Check sheet for the modelled part. Datum: model origin and axes. Units: mm. A direction names the side the tool comes from. Give positions to 0.01 mm unless a question says otherwise; leave off trailing zeros. Write each loop counter-clockwise with the first axis right and the second up, starting at its lowest first coordinate (ties: lowest second). Pieces come first, ordered by that corner, then holes. Notation, with made-up numbers: M 15.5,40 L 71.5,40 A32 cw 71.5,79 Z; hole C 19,48 d9. An arc over 180 degrees is marked long. Write item = value, one per line. Start each with the question number.
1) Sectioned sample at B-B, the plane y = 0. Record the cut outline in (x, z).
2) Scan lines: L1, parallel to Y at x = 0, z = 4.75; L2, parallel to Y at x = -4, z = -32; L3, parallel to Z at x = -3, y = -11.5. Record each from-to range of solid material in increasing order.
3) Gauge pin test, flat ends, axial feed: pin 1 (4 mm diameter, centred on y = -20, z = 0.5, fed in from -X); pin 2 (1.5 mm diameter, centred on y = -0.5, z = 4, fed in from -X); pin 3 (7.5 mm diameter, centred on x = -6, y = -20, fed in from +Z); pin 4 (10 mm diameter, centred on y = -34, z = -3, fed in from +X). Record the tip position at first contact, or that the pin passes through.
4) Set-up check for faces 1 (the face through (0.387, 12.494, 0.14)), 2 (the face through (-0.96, -56.07, 33.86)), 3 (the face through (0, -51, -30)), 4 (the face through (0, -15, 10)), 5 (the face through (10, -41, 1)): record each of +Z, -Z, +X, -X, +Y, -Y from which the full face is reachable in a straight line by a thin tool's end or side.
5) Draft check along Y on faces 6 (the face through (-7.493, 0.33, -0.14)), 7 (the face through (-10, -41, 1)), 8 (the face through (0, -51, 31)). Enter one of: pulls with the +Y half, pulls with the -Y half, needs draft (parallel to the pull), parting line crosses it, or undercut.
6) Sectioned sample at D-D, the plane z = 29.5. Record the cut outline in (x, y).
7) Sectioned sample at C-C, the plane z = 7. Record the cut outline in (x, y), then the cut area to 3 significant figures.
8) Sectioned sample at A-A, the plane x = 0. Record the cut outline in (y, z), then the cut area to 3 significant figures.
from build123d import *

# Parameters (mm, degrees)
SKETCH_1_R           = 12.5
SKETCH_1_R_2         = 7.5
EXTRUDE_1_DEPTH      = 10
EXTRUDE_3_DEPTH      = 10
EXTRUDE_4_REACH      = 66.833
EXTRUDE_4_END_RADIUS = 12.5
SKETCH_6_W           = 20
SKETCH_6_H           = 20
HOLE_WIZARD_M6_1_D   = 5


with BuildPart() as part:
    # Sketch 1 → Extrude 1 (new, symmetric)
    with BuildSketch(Plane.XY):
        Circle(SKETCH_1_R)
        Circle(SKETCH_1_R_2, mode=Mode.SUBTRACT)
    extrude(amount=EXTRUDE_1_DEPTH, both=True)



with BuildPart() as body_2:
    # Sketch 5 → Extrude 3 (new, symmetric)
    with BuildSketch(Plane(origin=(0, 0, 0), x_dir=(0, 0, -1), z_dir=(1, 0, 0))):
        with BuildLine():
            Line((21.657691454, -51), (41.168402769, -51))
            Line((41.168402769, -51), (41.168402769, -61))
            Line((41.168402769, -61), (-41.168402769, -61))
            Line((-41.168402769, -61), (-41.168402769, -51))
            Line((-41.168402769, -51), (-21.657691454, -51))
            Line((-21.657691454, -51), (-20, -51))
            ThreePointArc((-20, -51), (-12.928932188, -48.071067812), (-10, -41))
            Line((-10, -41), (-10, -12.5))
            Line((-10, -12.5), (10, -12.5))
            Line((10, -12.5), (10, -41))
            ThreePointArc((10, -41), (12.928932188, -48.071067812), (20, -51))
            Line((20, -51), (21.657691454, -51))
        make_face()
    extrude(amount=EXTRUDE_3_DEPTH, both=True)


with BuildPart() as part_1:
    add(part.part)

    add(body_2.part)  # Extrude 4 merges body 2
    # Extrude 4: up to this cylinder (the profile starts outside it)
    extrude_4_end = Plane(origin=(0, 0, 0), z_dir=(0, 0, -1)) * Cylinder(EXTRUDE_4_END_RADIUS, 159.666, mode=Mode.PRIVATE)
    # Sketch 6 → Extrude 4 (add, up to the surface)
    with BuildSketch(Plane(origin=(0, -12.5, 0), x_dir=(1, 0, 0), z_dir=(0, 1, 0)), mode=Mode.PRIVATE) as extrude_4_sk1:
        Rectangle(SKETCH_6_W, SKETCH_6_H)
    extrude_4_tool1 = extrude(extrude_4_sk1.sketch, amount=EXTRUDE_4_REACH, mode=Mode.PRIVATE) - extrude_4_end
    add(extrude_4_tool1.solids().sort_by_distance((0, -12.5, 0))[0])
    add(extrude_4_tool1.solids().sort_by_distance((0, -12.5, 0))[1])

    # Hole Wizard M6 _1 (through all)
    with Locations(Plane(origin=(0, -51, 36.168402769), x_dir=(0, 0, 1), z_dir=(0, 1, 0))):
        with Locations((0, 0)):
            hole_wizard_m6_1 = Hole(HOLE_WIZARD_M6_1_D / 2)

    # Mirror 1: Hole Wizard M6 _1 across plane
    add(hole_wizard_m6_1.mirror(Plane.XY), mode=Mode.SUBTRACT)


solid = part_1.part
Data:
q1.outline = M -12.5,-10 L -7.5,-10 L -7.5,10 L -12.5,10 Z; M 7.5,-10 L 12.5,-10 L 12.5,10 L 7.5,10 Z
q2.L1 = -61 to -7.5, 7.5 to 12.5
q2.L2 = -61 to -51
q2.L3 = -10 to 10
q3.pin_1 = -10
q3.pin_2 = -12.5
q3.pin_3 = 10
q3.pin_4 = 10
q4.face_1 = +Z, -Z
q4.face_2 = +Y, -Y
q4.face_3 = -Z, +X, -X, +Y
q4.face_4 = +Z, +X, -X, +Y
q4.face_5 = +Z, -Z, +X, -Y
q5.face_6 = undercut
q5.face_7 = needs draft
q5.face_8 = pulls with the +Y half
q6.outline = M -10,-61 L 10,-61 L 10,-51 L -10,-51 Z
q7.outline = M -10,-61 L 10,-61 L 10,-7.5 A12.5 ccw long -10,-7.5 Z; hole C 0,0 d15
q7.area = 1,310 mm2
q8.outline = M -61,-41.17 L -51,-41.17 L -51,-38.67 L -61,-38.67 Z; M -61,-33.67 L -51,-33.67 L -51,-20 A10 cw -41,-10 L -7.5,-10 L -7.5,10 L -41,10 A10 cw -51,20 L -51,33.67 L -61,33.67 Z; M -61,38.67 L -51,38.67 L -51,41.17 L -61,41.17 Z; M 7.5,-10 L 12.5,-10 L 12.5,10 L 7.5,10 Z
q8.area = 1,740 mm2
